Work out the finished part from the listing and answer in its coordinate system (mm). Face numbers are marked on the shaded views. A direction names the side the tool comes from. Give positions to 0.01 mm unless a question says otherwise; leave off trailing zeros. Loops run counter-clockwise (first coordinate to the right, second up) from the corner with the lowest first, then second, coordinate; pieces in that order, holes last. Notation, with made-up numbers: (-35.5, 46.5) - (4.5, 46.5) arc R10 ccw to (4.5, 51.5) - close; hole circle Ø10 at (-27.5, 25). An arc over 180 degrees is marked (long way). One line per question, with ' | ' between items. Start each with the question number.
1. Find the intervals of material crossed by line 1 (Y direction, x = 2.75, z = 2.6); line 2 (Z direction, x = 8, y = 0.1); line 3 (X direction, y = -2.6, z = -0.55), in increasing order.
2. Section A-A (x = 9.5) is taken. Determine the outline of the cut face in (y, z).
3. Each of these flat-tipped pins is pushed along its axis until it touches: pin 1 (3 mm diameter, centred on x = 17, z = -2, fed in from -Y); pin 2 (1 mm diameter, centred on x = 10, z = 1.5, fed in from -Y); pin 3 (3 mm diameter, centred on x = 10.5, z = -2.5, fed in from +Y). Where does it stop, or does it pass through?
4. Section B-B (x = 16.25) is taken. Determine the outline of the cut face in (y, z), plus the area to 3 significant figures.
5. Which of the six approach directions +Z, -Z, +X, -X, +Y, -Y give full straight-line access (tool end or side, diameter ignored) to the marked faces 1 and 2?
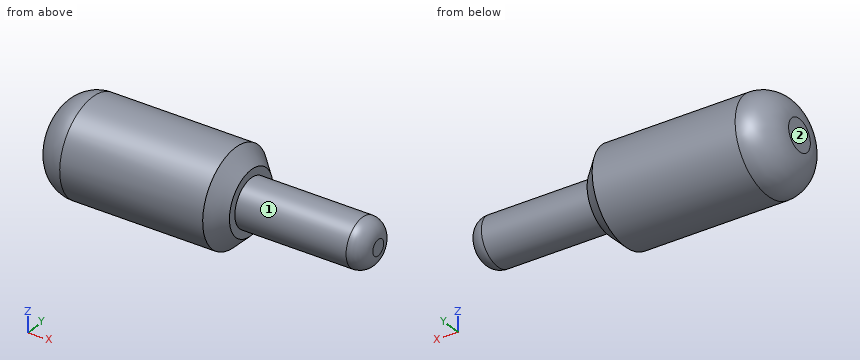
from build123d import *

# Parameters (mm, degrees)
FILLET1_R     = 2
FILLET2_R     = 1
CHAMFER1_SIZE = 1


with BuildPart() as part:
    # Sketch1 → Revolve1 (revolve)
    with BuildSketch(Plane.XY, mode=Mode.PRIVATE) as revolve1_sk:
        Polygon((0, 0), (0, 3), (12, 3), (12, 1.5), (20, 1.5), (20, 0), align=None)
    revolve(revolve1_sk.sketch.rotate(Axis((0, 0, 0), (1, 0, 0)), 90), axis=Axis((0, 0, 0), (1, 0, 0)))

    # Fillet1
    fillet1_edges = [part.edges().sort_by_distance(p)[0] for p in [
        (0, 0, -3),
    ]]
    fillet(fillet1_edges, radius=FILLET1_R)

    # Fillet2
    fillet2_edges = [part.edges().sort_by_distance(p)[0] for p in [
        (20, 0, -1.5),
    ]]
    fillet(fillet2_edges, radius=FILLET2_R)

    # Chamfer1
    chamfer1_edges = [part.edges().sort_by_distance(p)[0] for p in [
        (12, 0, -3),
    ]]
    chamfer(chamfer1_edges, length=CHAMFER1_SIZE)


solid = part.part
Conclusion:
1) line 1: -1.5 to 1.5 | line 2: -3 to 3 | line 3: 0.88 to 11.34
2) outline: circle Ø6 at (0, 0)
3) pin 1: y = -1.41 | pin 2: y = -2.83 | pin 3: y = 2.83
4) outline: circle Ø3 at (0, 0) | area: 7.07 mm²
5) face 1: +X | face 2: +Z, -Z, -X, +Y, -Y
